Input: part model. Units: mm. Frame: model coordinates. Give positions to 0.01 mm unless a question says otherwise; leave off trailing zeros. Write each loop counter-clockwise with the first axis right and the second up, starting at its lowest first coordinate (ties: lowest second). Pieces come first, ordered by that corner, then holes. Notation, with made-up numbers: (58, 62.5) - (86, 62.5) arc R19 cw to (86, 97.5) - close; hole circle Ø6 at (18, 22.5). An arc over 180 degrees is marked (long way). Answer as CSV lines item,"result".
```python
from build123d import *

# Parameters (mm, degrees)
SKETCH_1_W          = 59.5
SKETCH_1_H          = 86
EXTRUDE_1_DEPTH     = 6
SKETCH_2_R          = 1.75
CUT_EXTRUDE_1_DEPTH = 6
SKETCH_3_R          = 3
CUT_EXTRUDE_2_DEPTH = 3
FILLET_1_R          = 2


with BuildPart() as part:
    # 草图1 → 凸台-拉伸1 (new body)
    with BuildSketch(Plane.XY):
        Rectangle(SKETCH_1_W, SKETCH_1_H)
    extrude(amount=EXTRUDE_1_DEPTH)

    # 草图2 → 切除-拉伸1 (cut)
    with BuildSketch(Plane.XY.offset(6)):
        with Locations((-25, -39.5)):
            Circle(SKETCH_2_R)
        with Locations((25, -39.5)):
            Circle(SKETCH_2_R)
        with Locations((25, 39.5)):
            Circle(SKETCH_2_R)
        with Locations((-25, 39.5)):
            Circle(SKETCH_2_R)
        with Locations((-12.9, 15.8)):
            Circle(SKETCH_2_R)
        with Locations((9.727416998, -6.827416998)):
            Circle(SKETCH_2_R)
    extrude(amount=-CUT_EXTRUDE_1_DEPTH, mode=Mode.SUBTRACT)

    # 草图3 → 切除-拉伸2 (cut)
    with BuildSketch(Plane.XY.offset(6)):
        with Locations((-25, 39.5)):
            Circle(SKETCH_3_R)
        with Locations((25, 39.5)):
            Circle(SKETCH_3_R)
        with Locations((-12.9, 15.8)):
            Circle(SKETCH_3_R)
        with Locations((9.727416998, -6.827416998)):
            Circle(SKETCH_3_R)
        with Locations((-25, -39.5)):
            Circle(SKETCH_3_R)
        with Locations((25, -39.5)):
            Circle(SKETCH_3_R)
    extrude(amount=-CUT_EXTRUDE_2_DEPTH, mode=Mode.SUBTRACT)

    # 圆角1
    fillet_1_edges = [part.edges().sort_by_distance(p)[0] for p in [
        (29.75, -43, 3),
        (-29.75, -43, 3),
        (-29.75, 43, 3),
        (29.75, 43, 3),
    ]]
    fillet(fillet_1_edges, radius=FILLET_1_R)


solid = part.part
```
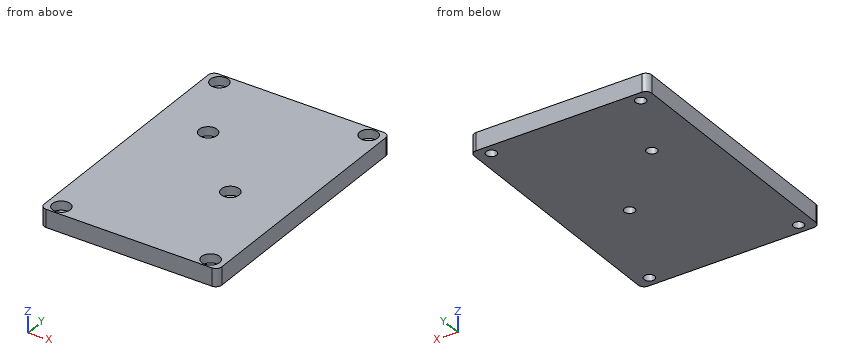
Item 1: Cut plane B-B on x = -25. Return the cut outline in (y, z).
The answers:
outline,"(-43, 0) - (-41.25, 0) - (-41.25, 3) - (-42.5, 3) - (-42.5, 6) - (-43, 6) - close; (-37.75, 0) - (37.75, 0) - (37.75, 3) - (36.5, 3) - (36.5, 6) - (-36.5, 6) - (-36.5, 3) - (-37.75, 3) - close; (41.25, 0) - (43, 0) - (43, 6) - (42.5, 6) - (42.5, 3) - (41.25, 3) - close"
Item 2: Cut plane D-D on y = 39.5. Return the cut outline in (x, z).
The answers:
outline,"(-29.75, 0) - (-26.75, 0) - (-26.75, 3) - (-28, 3) - (-28, 6) - (-29.75, 6) - close; (-23.25, 0) - (23.25, 0) - (23.25, 3) - (22, 3) - (22, 6) - (-22, 6) - (-22, 3) - (-23.25, 3) - close; (26.75, 0) - (29.75, 0) - (29.75, 6) - (28, 6) - (28, 3) - (26.75, 3) - close"
Item 3: Ray query, line 1 (Y direction, x = -25, z = 1.8); line 2 (Y direction, x = 25, z = 4.95); line 3 (Y direction, x = 9.5, z = 2.55). Return the intervals inside material, ascending. Write a range as from..to.
The answers:
line 1,"-43..-41.25, -37.75..37.75, 41.25..43"
line 2,"-43..-42.5, -36.5..36.5, 42.5..43"
line 3,"-43..-8.56, -5.09..43"
Item 4: Contact query for a flat-ended pin moving along its axis: pin 1 (1.8 mm diameter, centred on x = -12.5, y = 17, fed in from +Z). Output: stop coordinate, or through.
The answers:
pin 1,"z = 3"
Item 5: Cut plane A-A on y = 15.8. Return the cut outline in (x, z).
The answers:
outline,"(-29.75, 0) - (-14.65, 0) - (-14.65, 3) - (-15.9, 3) - (-15.9, 6) - (-29.75, 6) - close; (-11.15, 0) - (29.75, 0) - (29.75, 6) - (-9.9, 6) - (-9.9, 3) - (-11.15, 3) - close"
Item 6: Cut plane C-C on x = -12.9. Return the cut outline in (y, z).
The answers:
outline,"(-43, 0) - (14.05, 0) - (14.05, 3) - (12.8, 3) - (12.8, 6) - (-43, 6) - close; (17.55, 0) - (43, 0) - (43, 6) - (18.8, 6) - (18.8, 3) - (17.55, 3) - close"
